Geometry check sheet. Reference: drawing and pictorial views, mm from the part's lowest x, y, z. Round coordinates to 2 decimals unless told otherwise and drop trailing zeros. Write each loop counter-clockwise with the first axis right and the second up, starting at its lowest first coordinate (ties: lowest second). Pieces come first, ordered by that corner, then holes. Notation, with made-up numbers: (-17, -38.5) - (2, -38.5) arc R14 ccw to (2, -28.5) - close; hole circle Ø6 at (-21.5, -32.75). An arc over 180 degrees is marked (long way). Use one line per item in the form item = value. Start each with the question number.
1) Gauge pin test, flat end, axial feed: P1, Ø1.6, axis at y = 3, z = 3, coming from the +X side. Record the tip position at first contact, or that the pin passes through.
2) Section check A-A (z = 3). Record the boundary of the cut face in (x, y), then the cut area to 3 significant figures.
3) Section check D-D (y = 2). Record the boundary of the cut face in (x, z), then the cut area to 3 significant figures.
4) Scan lines: probe 1 along Y at (x, z) = (1.45, 3); probe 2 along Z at (x, y) = (0.3, 3.15); probe 3 along Z at (x, y) = (1, 0.95). Record each from-to range of solid material in increasing order.
5) Section check B-B (y = 3). Record the boundary of the cut face in (x, z), then the cut area to 3 significant figures.
6) Draft check along Z on the marked faces 1, 2, 3 and 4. Enter one of: +Z half, -Z half, draft (parallel to the pull), parting line (faces both ways), or undercut.
7) Section check C-C (x = 2.4). Record the boundary of the cut face in (y, z).
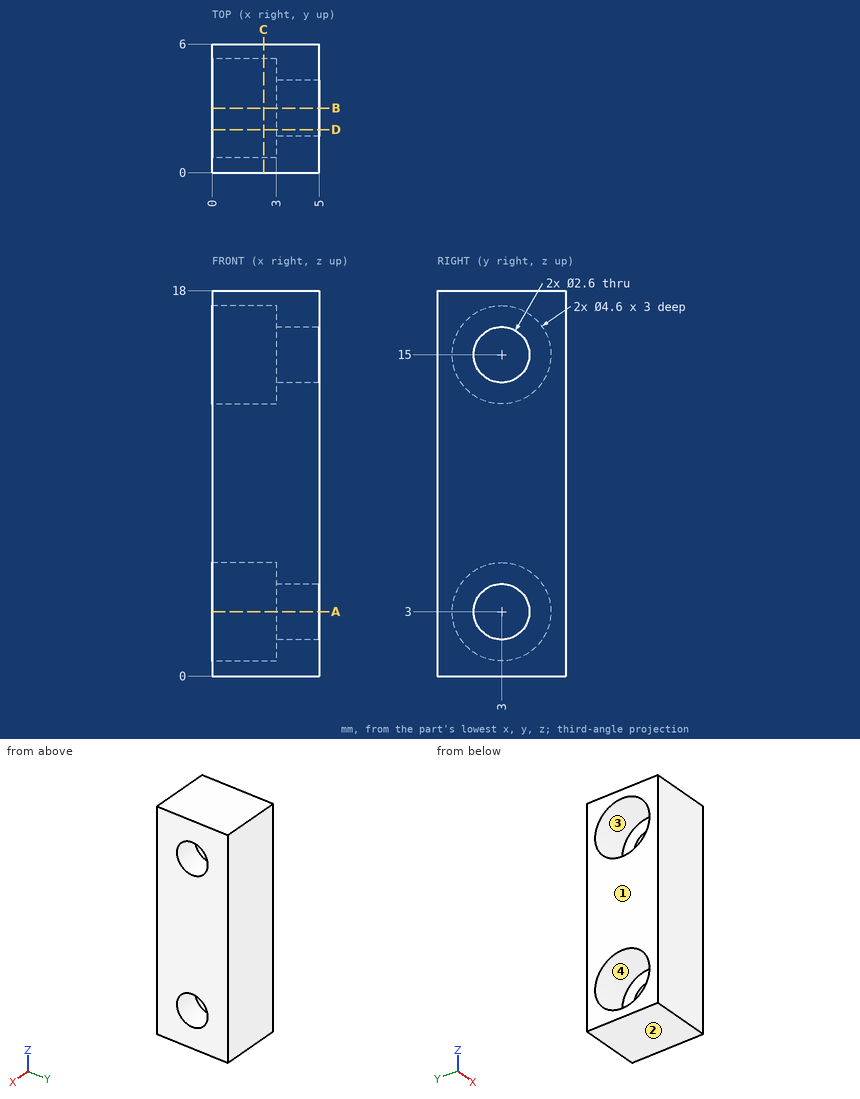
Results are:
q1.P1 = through
q2.outline = (0, 0) - (5, 0) - (5, 1.7) - (3, 1.7) - (3, 0.7) - (0, 0.7) - close; (0, 5.3) - (3, 5.3) - (3, 4.3) - (5, 4.3) - (5, 6) - (0, 6) - close
q2.area = 11.0 mm²
q3.outline = (0, 0) - (5, 0) - (5, 2.17) - (3, 2.17) - (3, 0.93) - (0, 0.93) - close; (0, 5.07) - (3, 5.07) - (3, 3.83) - (5, 3.83) - (5, 14.17) - (3, 14.17) - (3, 12.93) - (0, 12.93) - close; (0, 17.07) - (3, 17.07) - (3, 15.83) - (5, 15.83) - (5, 18) - (0, 18) - close
q3.area = 58.5 mm²
q4.probe_1 = 0 to 0.7, 5.3 to 6
q4.probe_2 = 0 to 0.7, 5.3 to 12.7, 17.3 to 18
q4.probe_3 = 0 to 1.96, 4.04 to 13.96, 16.04 to 18
q5.outline = (0, 0) - (5, 0) - (5, 1.7) - (3, 1.7) - (3, 0.7) - (0, 0.7) - close; (0, 5.3) - (3, 5.3) - (3, 4.3) - (5, 4.3) - (5, 13.7) - (3, 13.7) - (3, 12.7) - (0, 12.7) - close; (0, 17.3) - (3, 17.3) - (3, 16.3) - (5, 16.3) - (5, 18) - (0, 18) - close
q5.area = 52.0 mm²
q6.face_1 = draft
q6.face_2 = -Z half
q6.face_3 = undercut
q6.face_4 = undercut
q7.outline = (0, 0) - (6, 0) - (6, 18) - (0, 18) - close; hole circle Ø4.6 at (3, 3); hole circle Ø4.6 at (3, 15)
